from build123d import *

# Parameters (mm, degrees)
SKETCH_1_R          = 40
EXTRUDE_1_DEPTH     = 2
SKETCH_3_W          = 12
SKETCH_3_H          = 82
CUT_EXTRUDE_2_DEPTH = 2
CUT_EXTRUDE_3_DEPTH = 2


with BuildPart() as part:
    # 草图1 → 凸台-拉伸1 (new body)
    with BuildSketch(Plane.XY):
        Polygon((-367.770666468, 104.233847936), (-312.770666468, 104.233847936), (-312.770666468, 160.233847936), (682.229333532, 160.233847936), (682.229333532, 105.233847936), (737.229333532, 105.233847936), (737.229333532, -587.766152064), (682.229333532, -587.766152064), (682.229333532, -645.766152064), (-312.770666468, -645.766152064), (-312.770666468, -585.766152064), (-367.770666468, -585.766152064), align=None)
        with Locations((-217.770666468, 80.233847936)):
            Circle(SKETCH_1_R, mode=Mode.SUBTRACT)
        with Locations((587.229333532, 80.233847936)):
            Circle(SKETCH_1_R, mode=Mode.SUBTRACT)
    extrude(amount=EXTRUDE_1_DEPTH)

    # 草图3 → 切除-拉伸2 (cut)
    with BuildSketch(Plane(origin=(995.435508438, 654.453268367, 0), x_dir=(0, -1, 0), z_dir=(0, 0, -1))):
        with Locations((873.744003867, 950.143932906)):
            Rectangle(SKETCH_3_W, SKETCH_3_H)
    extrude(amount=-CUT_EXTRUDE_2_DEPTH, mode=Mode.SUBTRACT)

    # 草图4 → 切除-拉伸3 (cut)
    with BuildSketch(Plane(origin=(995.435508438, 654.453268367, 0), x_dir=(0, -1, 0), z_dir=(0, 0, -1))):
        Polygon((928.744003867, 949.143932916), (928.744003867, 909.143932916), (993.744003867, 909.143932916), (993.744003867, 949.143932916), (993.744003867, 994.143932916), (928.744003867, 994.143932916), align=None)
    extrude(amount=-CUT_EXTRUDE_3_DEPTH, mode=Mode.SUBTRACT)


solid = part.part
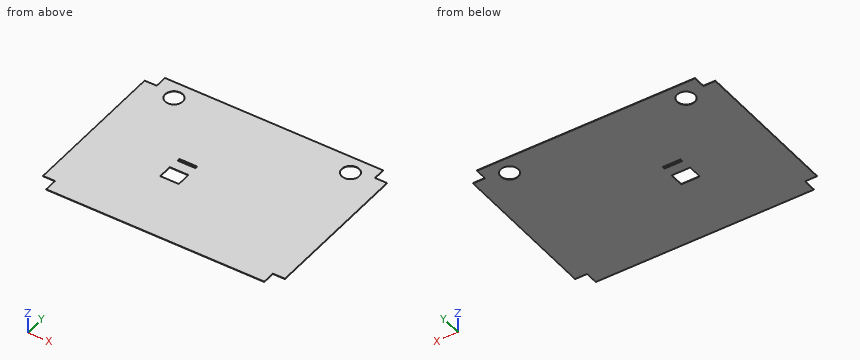
Check sheet for the modelled part. Datum: model origin and axes. Units: mm. Round coordinates to 2 decimals unless told otherwise and drop trailing zeros. Write each loop counter-clockwise with the first axis right and the second up, starting at its lowest first coordinate (ties: lowest second). Pieces come first, ordered by that corner, then holes. Notation, with made-up numbers: (71.25, 12.25) -> (127.25, 12.25) arc R30 ccw to (127.25, 35.25) -> close; hole circle Ø1 at (89.25, 21). An arc over 180 degrees is marked (long way). Answer as CSV lines item,"result". Start each with the question number.
1) Section check C-C on x = -231. Enter the section's corners in (y, z), and give its area (3 significant figures).
2) Section check A-A on x = 614.5. Enter the section's corners in (y, z), and give its area (3 significant figures).
3) Section check B-B on z = 0.5. Enter the section's corners in (x, y), and give its area (3 significant figures).
4) Go/stop test with flat-tipped pins: P1, Ø1, axis at x = -345.5, z = 1.5, coming from the -Y side; P2, Ø2, axis at x = -189.5, y = -512.5, coming from the -Z side; P3, Ø0.6, axis at y = 145, z = 1, coming from the +X side; P4, Ø0.6, axis at x = -342, z = 0.5, coming from the +Y side. Record where each tip stops, or that it passes through.
5) Material ranges on line 1 (X direction, y = -279, z = 0.6); line 2 (Y direction, x = 552.5, z = 1), recorded low to high. Write a range as from..to.
Found:
1,outline,"(-645.77, 0) -> (42.48, 0) -> (42.48, 2) -> (-645.77, 2) -> close; (117.98, 0) -> (160.23, 0) -> (160.23, 2) -> (117.98, 2) -> close"
1,area,"1,460 mm^2"
2,outline,"(-645.77, 0) -> (50.97, 0) -> (50.97, 2) -> (-645.77, 2) -> close; (109.5, 0) -> (160.23, 0) -> (160.23, 2) -> (109.5, 2) -> close"
2,area,"1,490 mm^2"
3,outline,"(-367.77, -585.77) -> (-312.77, -585.77) -> (-312.77, -645.77) -> (682.23, -645.77) -> (682.23, -587.77) -> (737.23, -587.77) -> (737.23, 105.23) -> (682.23, 105.23) -> (682.23, 160.23) -> (-312.77, 160.23) -> (-312.77, 104.23) -> (-367.77, 104.23) -> close; hole circle Ø80 at (-217.77, 80.23); hole (1.29, -339.29) -> (86.29, -339.29) -> (86.29, -274.29) -> (1.29, -274.29) -> close; hole (4.29, -225.29) -> (86.29, -225.29) -> (86.29, -213.29) -> (4.29, -213.29) -> close; hole circle Ø80 at (587.23, 80.23)"
3,area,"861,000 mm^2"
4,P1,"stops at y = -585.77"
4,P2,"stops at z = 0"
4,P3,"stops at x = 682.23"
4,P4,"stops at y = 104.23"
5,line 1,"x = -367.77..1.29, 86.29..737.23"
5,line 2,"y = -645.77..60.39, 100.08..160.23"
